Geometry: final body of the model. Coordinates: model frame, mm. Face numbers are marked on the shaded views. A direction names the side the tool comes from. Round coordinates to 2 decimals unless told otherwise and drop trailing zeros. Write each loop counter-clockwise with the first axis right and the second up, starting at its lowest first coordinate (ties: lowest second). Pieces come first, ordered by that corner, then holes. Notation, with made-up numbers: (43, 25) -> (71, 25) arc R16 ccw to (71, 49) -> close; hole circle Ø7 at (-36.5, 69.25). An arc over 180 degrees is marked (long way). Use one line per item in the form item = value. Start each with the question number.
1. Cut plane C-C, the plane y = 190. Return the cut outline in (x, z).
2. Cut plane B-B, the plane x = 0. Return the cut outline in (y, z), plus the area to 3 significant figures.
3. Line query: L1, parallel to Z at x = 0, y = 370; L2, parallel to Z at x = 0, y = 181; L3, parallel to Y at x = -29, z = 8.5. Output: solid intervals per line, ascending.
4. Pin query (flat end, axial travel): pin 1 Ø8 at (x, y) = (-2, 438.5) entering from +Z; pin 2 Ø12 at (x, y) = (-25.5, 542.5) entering from -Z; pin 3 Ø6 at (y, z) = (228.5, 27) entering from -X. Return the tip coordinate at first contact, or that it passes through.
5. Reachability of the marked faces 3 and 4 from +Z, -Z, +X, -X, +Y, -Y: full face, straight path, thin tool, end or side. Return the list, or none.
6. Cut plane A-A, the plane z = 0. Return the cut outline in (x, y), plus the area to 3 significant figures.
7. Draft query along Y for the marked faces 1 and 2. Return one class per face: pulls with the +Y half, pulls with the -Y half, needs draft (parallel to the pull), parting line crosses it, or undercut.
```python
from build123d import *

# Parameters (mm, degrees)
CUT_EXTRUDE1_REACH = 688.786
SKETCH2_R          = 20


with BuildPart() as part:
    # Sketch1 → Revolve1 (revolve)
    with BuildSketch(Plane.XY, mode=Mode.PRIVATE) as revolve1_sk:
        Polygon((0, 0), (35, 0), (35, 330), (30, 330), (30, 360), (29.5, 360), (29.5, 545), (30, 545), (30, 610), (25, 610), (25, 685), (0, 685), align=None)
    revolve(revolve1_sk.sketch.rotate(Axis((0, 685, 0), (0, -1, 0)), 180), axis=Axis((0, 685, 0), (0, -1, 0)))

    # Sketch2 → Cut-Extrude1 (cut, up to next)
    with BuildSketch(Plane(origin=(0, 685, 0), x_dir=(1, 0, 0), z_dir=(0, 1, 0)), mode=Mode.PRIVATE) as cut_extrude1_sk1:
        with Locations(Location((0, 0, 0), (0, 0, 180))):
            Circle(SKETCH2_R)
    cut_extrude1_tool1 = extrude(cut_extrude1_sk1.sketch, amount=-CUT_EXTRUDE1_REACH, mode=Mode.PRIVATE) & part.part
    add(cut_extrude1_tool1.solids().sort_by_distance((0, 685, 0))[0], mode=Mode.SUBTRACT)


solid = part.part
```
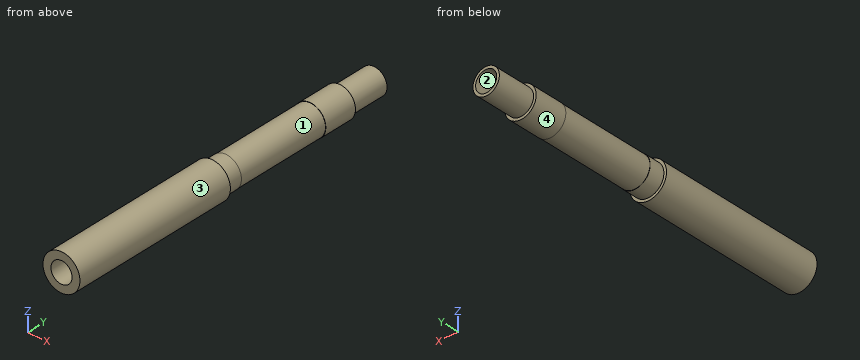
Outcome:
q1.outline = circle Ø70 at (0, 0); hole circle Ø40 at (0, 0)
q2.outline = (0, -35) -> (330, -35) -> (330, -30) -> (360, -30) -> (360, -29.5) -> (545, -29.5) -> (545, -30) -> (610, -30) -> (610, -25) -> (685, -25) -> (685, -20) -> (0, -20) -> close; (0, 20) -> (685, 20) -> (685, 25) -> (610, 25) -> (610, 30) -> (545, 30) -> (545, 29.5) -> (360, 29.5) -> (360, 30) -> (330, 30) -> (330, 35) -> (0, 35) -> close
q2.area = 16,100 mm^2
q3.L1 = -29.5 to -20, 20 to 29.5
q3.L2 = -35 to -20, 20 to 35
q3.L3 = 0 to 330
q4.pin_1 = 29.5
q4.pin_2 = -22.32
q4.pin_3 = -25.48
q5.face_3 = +Y, -Y
q5.face_4 = +Y
q6.outline = (-35, 0) -> (-20, 0) -> (-20, 685) -> (-25, 685) -> (-25, 610) -> (-30, 610) -> (-30, 545) -> (-29.5, 545) -> (-29.5, 360) -> (-30, 360) -> (-30, 330) -> (-35, 330) -> close; (20, 0) -> (35, 0) -> (35, 330) -> (30, 330) -> (30, 360) -> (29.5, 360) -> (29.5, 545) -> (30, 545) -> (30, 610) -> (25, 610) -> (25, 685) -> (20, 685) -> close
q6.area = 16,100 mm^2
q7.face_1 = undercut
q7.face_2 = needs draft
